The listing builds one solid part. Answer for the finished solid, in the listing's coordinates (mm). Face numbers are marked on the shaded views. A direction names the side the tool comes from. Coordinates: 2 decimals unless noted, no trailing zeros. Loops run counter-clockwise (first coordinate to the right, second up) from the corner with the lowest first, then second, coordinate; pieces in that order, holes last. Notation, with made-up numbers: M 39.25,52.25 L 82.25,52.25 A24 cw 82.25,77.25 Z; hole C 67,-2 d10. An arc over 180 degrees is marked long. Return JSON: item names as keys, results as strings. Group by question number.
1. Straight lines are drawn through the part: L1, parallel to X at y = 0, z = 7; L2, parallel to X at y = 15.5, z = -22; L3, parallel to Z at x = -9.35, y = 20. For each, find the intervals that lie inside material, in ascending order. Write a range as from..to.
2. Section B-B (x = -3.75) is taken. Write down the section's boundary in (y, z).
3. Which of the six approach directions +Z, -Z, +X, -X, +Y, -Y give full straight-line access (tool end or side, diameter ignored) to the marked faces 5 and 6?
4. Section A-A (y = 0) is taken. Write down the section's boundary in (x, z), then the cut area to 3 significant figures.
5. Given P1, Ø1.6, axis at x = -9.5, z = 22, coming from the -Y side (3 decimals); P2, Ø3, axis at x = 5.5, z = -21.5, coming from the +Y side; P3, Ø8, axis at y = 18.5, z = 12.5, coming from the +X side; P4, Ø3.5, axis at y = 20, z = -18, coming from the -X side, each flat-ended and moving along its own axis, determine where each tip first touches the part or whether it passes through.
6. The mould has two halves that part along X. Classify the marked faces 1, 2, 3 and 4: pulls with the +X half, pulls with the -X half, needs draft (parallel to the pull), parting line crosses it, or undercut.
```python
from build123d import *

# Parameters (mm, degrees)
SLEEVE_TUBE_PROFILE_R   = 12
SLEEVE_TUBE_PROFILE_R_2 = 10.5
SLEEVE_TUBE_24X60_DEPTH = 30
MOUNTING_LUGS_DEPTH     = 60
LUG_FILLET_R10_R        = 10
LUG_FILLET_R5_R         = 5
LUG_GAP_CUT_PROFILE_R   = 3
LUG_GAP_CUT_DEPTH       = 60
LUG_SLOTS_REACH         = 42.853
LUG_SLOTS_END_RADIUS    = 12


with BuildPart() as part:
    # Sleeve Tube Profile → Sleeve Tube Ø24x60 (new, symmetric)
    with BuildSketch(Plane.XY):
        Circle(SLEEVE_TUBE_PROFILE_R)
        Circle(SLEEVE_TUBE_PROFILE_R_2, mode=Mode.SUBTRACT)
    extrude(amount=SLEEVE_TUBE_24X60_DEPTH, both=True)

    # Mounting Lugs Profile → Mounting Lugs (add)
    with BuildSketch(Plane.XY.offset(30)):
        with BuildLine():
            Line((-8.5, 25), (-8.5, 8.470537173))
            ThreePointArc((-8.5, 8.470537173), (-9.295504635, 7.589044312), (-10, 6.633249581))
            Line((-10, 6.633249581), (-10, 25))
            Line((-10, 25), (-8.5, 25))
        make_face()
        with BuildLine():
            Line((10, 25), (10, 6.633249581))
            ThreePointArc((10, 6.633249581), (9.295504635, 7.589044312), (8.5, 8.470537173))
            Line((8.5, 8.470537173), (8.5, 25))
            Line((8.5, 25), (10, 25))
        make_face()
    extrude(amount=-MOUNTING_LUGS_DEPTH)

    # Lug Fillet R10
    lug_fillet_r10_edges = [part.edges().sort_by_distance(p)[0] for p in [
        (-10, 6.633249581, 0),
        (10, 6.633249581, 0),
    ]]
    fillet(lug_fillet_r10_edges, radius=LUG_FILLET_R10_R)

    # Lug Fillet R5
    lug_fillet_r5_edges = [part.edges().sort_by_distance(p)[0] for p in [
        (-9.25, 25, -30),
        (-9.25, 25, 30),
        (9.25, 25, -30),
        (9.25, 25, 30),
    ]]
    fillet(lug_fillet_r5_edges, radius=LUG_FILLET_R5_R)

    # Lug Gap Cut Profile → Lug Gap Cut (cut)
    with BuildSketch(Plane(origin=(10, 0, 0), x_dir=(0, 0, -1), z_dir=(1, 0, 0))):
        with Locations(Location((18, 20, 0), (0, 0, 90))):
            Circle(LUG_GAP_CUT_PROFILE_R)
        with BuildLine():
            Line((-25, 23), (-21, 23))
            ThreePointArc((-21, 23), (-18, 20), (-21, 17))
            Line((-21, 17), (-25, 17))
            ThreePointArc((-25, 17), (-28, 20), (-25, 23))
        make_face()
    extrude(amount=-LUG_GAP_CUT_DEPTH, mode=Mode.SUBTRACT)

    # Lug Slots: up to this cylinder (the profile starts inside it)
    lug_slots_end = Plane(origin=(0, 0, -24.504673), z_dir=(0, 0, -1)) * Cylinder(LUG_SLOTS_END_RADIUS, 110.706, mode=Mode.PRIVATE)
    # Lug Slots Profile → Lug Slots (cut, up to the surface)
    with BuildSketch(Plane(origin=(0, 0, 0), x_dir=(1, 0, 0), z_dir=(0, 1, 0)), mode=Mode.PRIVATE) as lug_slots_sk1:
        with BuildLine():
            Line((-2.25, 30), (-2.25, 22.75))
            ThreePointArc((-2.25, 22.75), (-1.590990258, 21.159009742), (0, 20.5))
            Line((0, 20.5), (5, 20.5))
            ThreePointArc((5, 20.5), (7.25, 22.75), (5, 25))
            Line((5, 25), (2.25, 25))
            Line((2.25, 25), (2.25, 30))
            Line((2.25, 30), (-2.25, 30))
        make_face()
    lug_slots_tool1 = extrude(lug_slots_sk1.sketch, amount=-LUG_SLOTS_REACH, mode=Mode.PRIVATE) & lug_slots_end
    add(lug_slots_tool1.solids().sort_by_distance((1.518168, 0, -24.504673))[0], mode=Mode.SUBTRACT)


solid = part.part
```
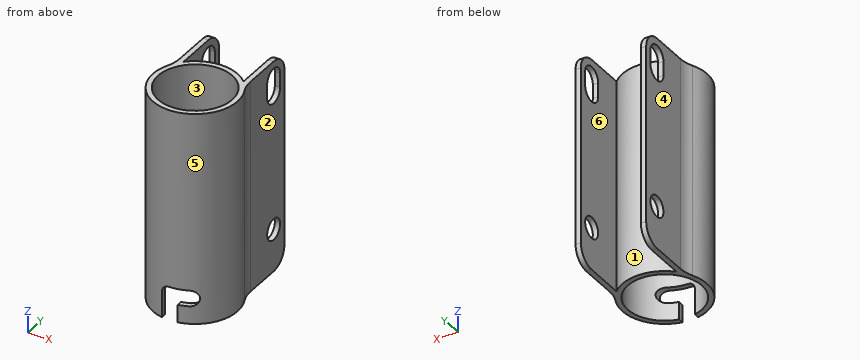
Worked out:
{
 "1": {"L1": "-12..-10.5, 10.5..12", "L2": "-10..-8.5, 8.5..10", "L3": "-30..-21, -15..18, 28..30"},
 "2": {"outline": "M -11.4,-30 L -9.81,-30 L -9.81,30 L -11.4,30 Z; M 9.81,-30 L 11.4,-30 L 11.4,30 L 9.81,30 Z"},
 "3": {"face 5": "+Z, -Z", "face 6": "+Z, -Z, +Y"},
 "4": {"outline": "M -12,-30 L -10.5,-30 L -10.5,30 L -12,30 Z; M 10.5,-30 L 12,-30 L 12,30 L 10.5,30 Z", "area": "180 mm^2"},
 "5": {"P1": "y = -8.265", "P2": "y = 11.31", "P3": "x = 10", "P4": "through"},
 "6": {"face 1": "undercut", "face 2": "pulls with the +X half", "face 3": "undercut", "face 4": "pulls with the -X half"}
}
